from build123d import *

# Parameters (mm, degrees)
HOUSING_BLOCK_DEPTH           = 40
TOP_LUG_SKETCH_R              = 5
TOP_LUG_DEPTH                 = 15
BASE_FLANGE_SKETCH_W          = 70
BASE_FLANGE_SKETCH_H          = 50.64236497
BASE_FLANGE_DEPTH             = 25
BEARING_SEAT_CUT_DEPTH        = 80
FLANGE_END_ROUND_R20_A_R      = 20
FLANGE_END_ROUND_R20_B_R      = 20
MOUNTING_HOLES_SET_1_SKETCH_R = 5
MOUNTING_HOLES_SET_1_DEPTH    = 25
MOUNTING_HOLES_SET_2_SKETCH_R = 5
MOUNTING_HOLES_SET_2_DEPTH    = 25
SUPPORT_RIB_1_REACH           = 115.578
SUPPORT_RIB_1_SKETCH_WALL_W   = 264.511672892
SUPPORT_RIB_1_SKETCH_WALL_H   = 10
SUPPORT_RIB_2_REACH           = 115.578
SUPPORT_RIB_2_SKETCH_WALL_W   = 264.511672892
SUPPORT_RIB_2_SKETCH_WALL_H   = 10


with BuildPart() as part:
    # Housing Block Sketch → Housing Block (new, symmetric)
    with BuildSketch(Plane.XY):
        with BuildLine():
            Line((-40, 0), (-25, 0))
            ThreePointArc((-25, 0), (0, 25), (25, 0))
            Line((25, 0), (40, 0))
            ThreePointArc((40, 0), (0, 40), (-40, 0))
        make_face()
    extrude(amount=HOUSING_BLOCK_DEPTH, both=True)

    # Top Lug Sketch → Top Lug (add, symmetric)
    with BuildSketch(Plane.XY):
        with BuildLine():
            Line((-20, 50), (-20, 34.002392221))
            Line((-20, 34.002392221), (20, 34.641016151))
            Line((20, 34.641016151), (20, 50))
            ThreePointArc((20, 50), (0, 70), (-20, 50))
        make_face()
        with Locations((0, 50)):
            Circle(TOP_LUG_SKETCH_R, mode=Mode.SUBTRACT)
    extrude(amount=TOP_LUG_DEPTH, both=True)

    # Base Flange Sketch → Base Flange (add)
    with BuildSketch(Plane(origin=(0, 0, 0), x_dir=(1, 0, 0), z_dir=(0, 1, 0))):
        with Locations((45, 0)):
            Rectangle(BASE_FLANGE_SKETCH_W, BASE_FLANGE_SKETCH_H)
        with Locations((-45, 0)):
            Rectangle(BASE_FLANGE_SKETCH_W, BASE_FLANGE_SKETCH_H)
    extrude(amount=BASE_FLANGE_DEPTH)

    # Bearing Seat Sketch → Bearing Seat Cut (cut)
    with BuildSketch(Plane.XY.offset(25.321182485)):
        with BuildLine():
            Line((-10, 22.912878475), (-10, 0))
            Line((-10, 0), (-25, 0))
            ThreePointArc((-25, 0), (-20.916500663, 13.693063938), (-10, 22.912878475))
        make_face()
        with BuildLine():
            Line((10, 22.912878475), (10, 0))
            Line((10, 0), (25, 0))
            ThreePointArc((25, 0), (20.916500663, 13.693063938), (10, 22.912878475))
        make_face()
    extrude(amount=-BEARING_SEAT_CUT_DEPTH, mode=Mode.SUBTRACT)

    # Flange End Round R20 A
    flange_end_round_r20_a_edges = [part.edges().sort_by_distance(p)[0] for p in [
        (80, 12.5, -25.321182485),
        (80, 12.5, 25.321182485),
        (-80, 12.5, 25.321182485),
    ]]
    fillet(flange_end_round_r20_a_edges, radius=FLANGE_END_ROUND_R20_A_R)

    # Flange End Round R20 B
    flange_end_round_r20_b_edges = [part.edges().sort_by_distance(p)[0] for p in [
        (-80, 12.5, -25.321182485),
    ]]
    fillet(flange_end_round_r20_b_edges, radius=FLANGE_END_ROUND_R20_B_R)

    # Mounting Holes Set 1 Sketch → Mounting Holes Set 1 (cut)
    with BuildSketch(Plane(origin=(0, 25, 0), x_dir=(1, 0, 0), z_dir=(0, 1, 0))):
        with Locations(Location((-60, 8.824452572, 0), (0, 0, 270))):
            Circle(MOUNTING_HOLES_SET_1_SKETCH_R)
        with Locations(Location((-60, -11.175547428, 0), (0, 0, 270))):
            Circle(MOUNTING_HOLES_SET_1_SKETCH_R)
    extrude(amount=-MOUNTING_HOLES_SET_1_DEPTH, mode=Mode.SUBTRACT)

    # Mounting Holes Set 2 Sketch → Mounting Holes Set 2 (cut)
    with BuildSketch(Plane(origin=(0, 25, 0), x_dir=(1, 0, 0), z_dir=(0, 1, 0))):
        with Locations(Location((60, 11.288668944, 0), (0, 0, 270))):
            Circle(MOUNTING_HOLES_SET_2_SKETCH_R)
        with Locations(Location((60, -8.711331056, 0), (0, 0, 270))):
            Circle(MOUNTING_HOLES_SET_2_SKETCH_R)
    extrude(amount=-MOUNTING_HOLES_SET_2_DEPTH, mode=Mode.SUBTRACT)

    # Support Rib 1 Sketch wall → Support Rib 1 (add, up to next)
    with BuildSketch(Plane(origin=(-32.5, 37.5, 0), x_dir=(-0.707106781187, -0.707106781187, 0), z_dir=(0.707106781187, -0.707106781187, 0)), mode=Mode.PRIVATE) as support_rib_1_sk1:
        Rectangle(SUPPORT_RIB_1_SKETCH_WALL_W, SUPPORT_RIB_1_SKETCH_WALL_H)
    support_rib_1_tool1 = extrude(support_rib_1_sk1.sketch, amount=SUPPORT_RIB_1_REACH, mode=Mode.PRIVATE) - part.part
    add(support_rib_1_tool1.solids().sort_by_distance((-32.5, 37.5, 0))[0])

    # Support Rib 2 Sketch wall → Support Rib 2 (add, up to next)
    with BuildSketch(Plane(origin=(32.5, 37.5, 0), x_dir=(0.707106781187, -0.707106781187, 0), z_dir=(0.707106781187, 0.707106781187, 0)), mode=Mode.PRIVATE) as support_rib_2_sk1:
        Rectangle(SUPPORT_RIB_2_SKETCH_WALL_W, SUPPORT_RIB_2_SKETCH_WALL_H)
    support_rib_2_tool1 = extrude(support_rib_2_sk1.sketch, amount=-SUPPORT_RIB_2_REACH, mode=Mode.PRIVATE) - part.part
    add(support_rib_2_tool1.solids().sort_by_distance((32.5, 37.5, 0))[0])


solid = part.part
CAD build for the part. Positions are in the model's coordinates, mm. A direction names the side the tool comes from. Round coordinates to 2 decimals unless told otherwise and drop trailing zeros. Order: outer loops, then holes, each group sorted by start corner. A loop starts at its lowest first (then second) coordinate and runs counter-clockwise, first axis right, second up. Notation, with made-up numbers: (78.5, 76.25) - (118.5, 76.25) arc R16 ccw to (118.5, 94.25) - close; hole circle Ø8 at (59.25, 54). An arc over 180 degrees is marked (long way). Return JSON: item names as keys, results as strings.
(1) Cut at C-C (y = 9). Give the cut face in (x, z), then the cut area to 3 significant figures.
Answer key:
{"outline": "(-80, -5.32) arc R20 ccw to (-60, -25.32) - (-38.97, -25.32) - (-38.97, -40) - (-23.32, -40) - (-23.32, 40) - (-38.97, 40) - (-38.97, 25.32) - (-60, 25.32) arc R20 ccw to (-80, 5.32) - close; (23.32, -40) - (38.97, -40) - (38.97, -25.32) - (60, -25.32) arc R20 ccw to (80, -5.32) - (80, 5.32) arc R20 ccw to (60, 25.32) - (38.97, 25.32) - (38.97, 40) - (23.32, 40) - close; hole circle Ø10 at (-60, -8.82); hole circle Ø10 at (-60, 11.18); hole circle Ø10 at (60, -11.29); hole circle Ø10 at (60, 8.71)", "area": "6,000 mm^2"}
(2) Pull direction Z, two halves, no side cores. Call faces 1 (the face through (0, 56, -15)), 2 (the face through (55, 25, 0)), 3 (the face through (64.216, 12.675, -8.601)): +Z half, -Z half, draft (parallel to the pull), parting line (faces both ways), or undercut.
Answer key:
{"face 1": "-Z half", "face 2": "draft", "face 3": "undercut"}
(3) Tool access for faces 4 (the face through (49, 12, 25.321)), 5 (the face through (-20, 42, 10)), 6 (the face through (-29, 35, -5)): list every direction of +Z, -Z, +X, -X, +Y, -Y with a clear straight run to the whole face (end or side of a thin tool).
Answer key:
{"face 4": "+Z, +X, +Y", "face 5": "+Z, -X, +Y", "face 6": "-Z, -X, +Y"}
(4) Cut at B-B (z = 11). Give the cut face in (x, y).
Answer key:
{"outline": "(-79.18, 0) - (-65, 0) - (-65, 25) - (-79.18, 25) - close; (-55, 0) - (-25, 0) arc R25 cw to (25, 0) - (55.55, 0) - (55.55, 25) - (31.22, 25) arc R40 ccw to (20, 34.64) - (20, 50) arc R20 ccw to (-20, 50) - (-20, 34.64) arc R40 ccw to (-31.22, 25) - (-55, 25) - close; (64.45, 0) - (79.18, 0) - (79.18, 25) - (64.45, 25) - close; hole circle Ø10 at (0, 50)"}
(5) Wall check: probe 1 along Y at (x, z) = (0, 2); probe 2 along X at (y, z) = (50.5, 7.5); probe 3 along Z at (x, y) = (64, 21). Give the ranges that are in metal, low to high. Write a range as from..to.
Answer key:
{"probe 1": "y = 25..45, 55..70", "probe 2": "x = -19.99..-4.97, 4.97..19.99", "probe 3": "z = -24.92..-14.29, -8.29..5.71, 11.71..24.92"}
(6) Cut at A-A (x = 0). Give the cut face in (y, z).
Answer key:
{"outline": "(25, -40) - (40, -40) - (40, -15) - (45, -15) - (45, 15) - (40, 15) - (40, 40) - (25, 40) - close; (55, -15) - (70, -15) - (70, 15) - (55, 15) - close"}
(7) Pin check, flat tips, straight feed: pin 1 Ø1 at (x, z) = (3.5, -30) entering from -Y; pin 2 Ø3 at (x, y) = (-51.5, 14.5) entering from -Z; pin 3 Ø11.5 at (x, y) = (0, 50) entering from -Z. Stop position of each tip, or through.
Answer key:
{"pin 1": "stops at y = 24.68", "pin 2": "stops at z = -25.32", "pin 3": "stops at z = -15"}
(8) Cut at D-D (z = 23). Give the cut face in (x, y).
Answer key:
{"outline": "(-69.35, 0) - (-25, 0) arc R25 cw to (25, 0) - (69.35, 0) - (69.35, 25) - (31.22, 25) arc R40 ccw to (-31.22, 25) - (-69.35, 25) - close"}
